Read the model definition and answer for the solid it produces. Units are mm, in the model's axes. A direction names the side the tool comes from. Round coordinates to 2 decimals unless told otherwise and drop trailing zeros. Loops run counter-clockwise (first coordinate to the right, second up) from the corner with the lowest first, then second, coordinate; pieces in that order, holes last. Notation, with made-up numbers: M -40,50 L -27,50 A18 ccw -27,63 Z; hole C 22,56 d11. An arc over 180 degrees is marked long. Write each question's results on one line, items separated by ' | '.
```python
from build123d import *

# Parameters (mm, degrees)
CLAMP_RING_SKETCH_R             = 48
CLAMP_RING_96_DEPTH             = 40
CLAMP_START                     = -40
CLAMP_LUG_DEPTH                 = 40
CLAMP_BORE_AND_SPLIT_SLOT_DEPTH = 40
PIVOT_EYE_SKETCH_R              = 26
PIVOT_EYE_52_DEPTH              = 40
CONNECTING_START                = -40
CONNECTING_ARM_DEPTH            = 40
ARM_RIB_A_DEPTH                 = 16
ARM_RIB_B_DEPTH                 = 16
PIVOT_BORE_SKETCH_R             = 14
PIVOT_BORE_28_DEPTH             = 40
CLAMP_SCREW_HOLE_SKETCH_R       = 5
CLAMP_SCREW_HOLE_10_DEPTH       = 80


with BuildPart() as part:
    # Clamp Ring Sketch → Clamp Ring Ø96 (new body)
    with BuildSketch(Plane.XY):
        Circle(CLAMP_RING_SKETCH_R)
    extrude(amount=CLAMP_RING_96_DEPTH)

    # Clamp Lug Sketch → Clamp Lug (add)
    with BuildSketch(Plane.XY.offset(40).offset(CLAMP_START)):
        with BuildLine():
            Line((30, -67.46998799), (30, -37.46998799))
            ThreePointArc((30, -37.46998799), (0, -48), (-30, -37.46998799))
            Line((-30, -37.46998799), (-30, -67.46998799))
            Line((-30, -67.46998799), (30, -67.46998799))
        make_face()
    extrude(amount=CLAMP_LUG_DEPTH)

    # Clamp Bore and Split Sketch → Clamp Bore and Split Slot (cut)
    with BuildSketch(Plane.XY.offset(40)):
        with BuildLine():
            Line((-3, -67.46998799), (3, -67.46998799))
            Line((3, -67.46998799), (3, -31.859064644))
            ThreePointArc((3, -31.859064644), (0, 32), (-3, -31.859064644))
            Line((-3, -31.859064644), (-3, -67.46998799))
        make_face()
    extrude(amount=-CLAMP_BORE_AND_SPLIT_SLOT_DEPTH, mode=Mode.SUBTRACT)



with BuildPart() as body_2:
    # Pivot Eye Sketch → Pivot Eye Ø52 (new body)
    with BuildSketch(Plane.XY.offset(40)):
        with Locations((110, 0)):
            Circle(PIVOT_EYE_SKETCH_R)
    extrude(amount=-PIVOT_EYE_52_DEPTH)


with BuildPart() as part_1:
    add(part.part)

    add(body_2.part)  # Connecting Arm merges body 2
    # Connecting Arm Sketch → Connecting Arm (add)
    with BuildSketch(Plane.XY.offset(40).offset(CONNECTING_START)):
        with BuildLine():
            Line((47.623523599, 6), (84.701778719, 6))
            ThreePointArc((84.701778719, 6), (84, 0), (84.701778719, -6))
            Line((84.701778719, -6), (47.623523599, -6))
            ThreePointArc((47.623523599, -6), (48, 0), (47.623523599, 6))
        make_face()
    extrude(amount=CONNECTING_ARM_DEPTH)

    # Arm Rib A Sketch → Arm Rib A (add)
    with BuildSketch(Plane(origin=(0, 6, 0), x_dir=(1, 0, 0), z_dir=(0, 1, 0))):
        Polygon((98.516804154, -14), (110.350889359, -14), (110.350889359, -26), (98.516804154, -26), (39.268352847, -26), (39.268352847, -20), (39.268352847, -14), align=None)
    extrude(amount=ARM_RIB_A_DEPTH)

    # Arm Rib B Sketch → Arm Rib B (add)
    with BuildSketch(Plane.XZ.offset(6)):
        Polygon((38.239733901, 20), (38.239733901, 26), (110.350889359, 26), (110.350889359, 14), (38.239733901, 14), align=None)
    extrude(amount=ARM_RIB_B_DEPTH)

    # Pivot Bore Sketch → Pivot Bore Ø28 (cut)
    with BuildSketch(Plane.XY.offset(40)):
        with Locations((110, 0)):
            Circle(PIVOT_BORE_SKETCH_R)
    extrude(amount=-PIVOT_BORE_28_DEPTH, mode=Mode.SUBTRACT)

    # Clamp Screw Hole Sketch → Clamp Screw Hole Ø10 (cut)
    with BuildSketch(Plane(origin=(30, 0, 0), x_dir=(0, 0, -1), z_dir=(1, 0, 0))):
        with Locations(Location((-20, -53.46998799, 0), (0, 0, 270))):
            Circle(CLAMP_SCREW_HOLE_SKETCH_R)
    extrude(amount=-CLAMP_SCREW_HOLE_10_DEPTH, mode=Mode.SUBTRACT)


solid = part_1.part
```
1. Determine the mould class of faces 1 (the face through (3, -46, 20)), 2 (the face through (16.69, -52.39, 24.88)), 3 (the face through (66, -6, 7)) for opening direction Y: released by +Y, released by -Y, zero draft, split by the parting line, or undercut.
Completed:
face 1: zero draft | face 2: undercut | face 3: released by -Y
2. Find the intervals of material crossed by L1, parallel to X at y = -0.5, z = 14.5; L2, parallel to X at y = -3, z = 7; L3, parallel to Y at x = 24, z = 16, in increasing order.
Completed:
L1: x = -48 to -32, 32 to 96.01, 123.99 to 136 | L2: x = -47.91 to -31.86, 31.86 to 96.33, 123.67 to 135.83 | L3: y = -67.47 to -56.47, -50.47 to -21.17, 21.17 to 41.57
3. Find section B-B, the plane x = 110. Give the vertices of the cut face in (y, z), then the cut area to 3 significant figures.
Completed:
outline: M -26,0 L -14,0 L -14,40 L -26,40 Z; M 14,0 L 26,0 L 26,40 L 14,40 Z | area: 960 mm2
4. Find section D-D, the plane z = 34.5. Give the vertices of the cut face in (x, y), then the cut area to 3 significant figures.
Completed:
outline: M -30,-67.47 L -3,-67.47 L -3,-31.86 A32 cw long 3,-31.86 L 3,-67.47 L 30,-67.47 L 30,-37.47 A48 ccw 47.62,-6 L 84.7,-6 A26 ccw long 84.7,6 L 47.62,6 A48 ccw long -30,-37.47 Z; hole C 110,0 d28 | area: 7,120 mm2
5. Given P1, Ø12, axis at x = 60.5, z = 26, coming from the +Y side; P2, Ø9.5, axis at x = 81.5, z = 20, coming from the -Y side; P3, Ø5, axis at y = 15.5, z = 5, coming from the +X side; P4, Ø17.5, axis at x = 71, y = -13, coming from the +Z side, each flat-ended and moving along its own axis, determine where each tip first touches the part or whether it passes through.
Completed:
P1: stops at y = 22 | P2: stops at y = -22 | P3: stops at x = 132.52 | P4: stops at z = 40
6. Which of the six approach directions +Z, -Z, +X, -X, +Y, -Y give full straight-line access (tool end or side, diameter ignored) to faces 4 (the face through (70, 14, 14)), 5 (the face through (70, 22, 20)), 6 (the face through (66, 6, 33))?
Completed:
face 4: -Z, +Y | face 5: +Z, -Z, +Y | face 6: +Z, +Y
7. Find section C-C, the plane y = 0. Give the vertices of the cut face in (x, z), then the cut area to 3 significant figures.
Completed:
outline: M -48,0 L -32,0 L -32,40 L -48,40 Z; M 32,0 L 96,0 L 96,40 L 32,40 Z; M 124,0 L 136,0 L 136,40 L 124,40 Z | area: 3,680 mm2
8. Find section A-A, the plane z = 20. Give the vertices of the cut face in (x, y).
Completed:
outline: M -30,-67.47 L -3,-67.47 L -3,-58.47 L -30,-58.47 Z; M -30,-48.47 L -3,-48.47 L -3,-31.86 A32 cw long 3,-31.86 L 3,-48.47 L 30,-48.47 L 30,-37.47 A48 ccw 42.66,-22 L 96.14,-22 A26 ccw long 96.14,22 L 42.66,22 A48 ccw long -30,-37.47 Z; M 3,-67.47 L 30,-67.47 L 30,-58.47 L 3,-58.47 Z; hole C 110,0 d28
